from build123d import *

# Parameters (mm, degrees)
EXTRUDE_1_DEPTH           = 20
HOLE_WIZARD_1_D           = 5.5
HOLE_WIZARD_1_DEPTH       = 14
HOLE_WIZARD_1_CBORE_D     = 10
HOLE_WIZARD_1_CBORE_DEPTH = 5.7
HOLE_WIZARD_1_TIP         = 1.652366702
HOLE_WIZARD_M5_1_D        = 4.2
HOLE_WIZARD_M5_1_DEPTH    = 14
HOLE_WIZARD_M5_1_TIP      = 1.2618073


with BuildPart() as part:
    # 草图1 → 凸台-拉伸1 (new, symmetric)
    with BuildSketch(Plane.XY):
        Polygon((0, 0), (450, 0), (450, 10), (38, 10), (38, 15), (18, 15), (0, 5), align=None)
    extrude(amount=EXTRUDE_1_DEPTH, both=True)

    # 打孔尺寸(%根据)内六角圆柱头螺钉的类型1
    with Locations(Plane(origin=(0, 10, 0), x_dir=(1, 0, 0), z_dir=(0, 1, 0))):
        with Locations((50, 12.5), (80, 12.5), (50, -12.5), (80, -12.5), (380, -12.5), (410, -12.5), (380, 12.5), (410, 12.5)):
            CounterBoreHole(HOLE_WIZARD_1_D / 2, HOLE_WIZARD_1_CBORE_D / 2, HOLE_WIZARD_1_CBORE_DEPTH, depth=HOLE_WIZARD_1_DEPTH)
            with Locations((0, 0, -(HOLE_WIZARD_1_DEPTH + HOLE_WIZARD_1_TIP / 2))):  # 118° drill point
                Cone(0, HOLE_WIZARD_1_D / 2, HOLE_WIZARD_1_TIP, mode=Mode.SUBTRACT)

    # M5 螺纹孔1
    with Locations(Plane(origin=(450, 0, 0), x_dir=(0, 0, -1), z_dir=(1, 0, 0))):
        with Locations((-12.5, 5), (12.5, 5)):
            Hole(HOLE_WIZARD_M5_1_D / 2, depth=HOLE_WIZARD_M5_1_DEPTH)
            with Locations((0, 0, -(HOLE_WIZARD_M5_1_DEPTH + HOLE_WIZARD_M5_1_TIP / 2))):  # 118° drill point
                Cone(0, HOLE_WIZARD_M5_1_D / 2, HOLE_WIZARD_M5_1_TIP, mode=Mode.SUBTRACT)


solid = part.part
CAD build for the part. Positions are in the model's coordinates, mm. A direction names the side the tool comes from. Coordinates: 2 decimals unless noted, no trailing zeros. Write each loop counter-clockwise with the first axis right and the second up, starting at its lowest first coordinate (ties: lowest second). Pieces come first, ordered by that corner, then holes. Notation, with made-up numbers: M 78.5,-38.75 L 112.5,-38.75 A23 cw 112.5,-11.75 Z; hole C 31.5,-33.75 d5. An arc over 180 degrees is marked long. Answer as a JSON object with one key per item and string values. Group by question number.
1) Pin check, flat tips, straight feed: pin 1 Ø8 at (x, z) = (52, 13.5) entering from +Y; pin 2 Ø5 at (x, z) = (381, -12.5) entering from +Y; pin 3 Ø3.5 at (x, z) = (380, -12.5) entering from +Y; pin 4 Ø1.5 at (y, z) = (13, 6) entering from +X. Stop position of each tip, or through.
2) Mould opens along Z. For faces 1 (the face through (222, 6, 20)), 2 (the face through (28, 15, 0)), 3 (the face through (412, 4.3, 15)) say: +Z half, -Z half, draft (parallel to the pull), parting line (faces both ways), or undercut.
3) Saw through at B-B (x = 420.5). Write the cut outline in (y, z).
4) Wall check: line 1 (Z direction, x = 441, y = 5); line 2 (Z direction, x = 410, y = 6.75); line 3 (X direction, y = 2.75, z = -13). Give the ranges that are in metal, low to high. Write a range as from..to.
5) Saw through at A-A (z = 2). Write the cut outline in (x, y), plus the area to 3 significant figures.
6) Tool access for faces 4 (the face through (9, 10, 0)), 5 (the face through (82, 4.3, -10)), 6 (the face through (247, 10, 0)): list every direction of +Z, -Z, +X, -X, +Y, -Y with a clear straight run to the whole face (end or side of a thin tool).
Values follow:
{
 "1": {"pin 1": "stops at y = 10", "pin 2": "stops at y = 4.3", "pin 3": "passes through", "pin 4": "stops at x = 38"},
 "2": {"face 1": "+Z half", "face 2": "draft", "face 3": "undercut"},
 "3": {"outline": "M 0,-20 L 10,-20 L 10,20 L 0,20 Z"},
 "4": {"line 1": "z = -20..-14.6, -10.4..10.4, 14.6..20", "line 2": "z = -20..-17.5, -7.5..7.5, 17.5..20", "line 3": "x = 0..47.3, 52.7..77.3, 82.7..377.3, 382.7..407.3, 412.7..450"},
 "5": {"outline": "M 0,0 L 450,0 L 450,10 L 38,10 L 38,15 L 18,15 L 0,5 Z", "area": "4,600 mm2"},
 "6": {"face 4": "+Z, -Z, -X, +Y", "face 5": "+Y", "face 6": "+Z, -Z, +X, +Y"}
}
